Design review of the part shown in the three views and the two pictorial views. Dimensions are in mm from the part's minimum x, y and z. A direction names the side the tool comes from. Coordinates: 2 decimals unless noted, no trailing zeros. Loops run counter-clockwise (first coordinate to the right, second up) from the corner with the lowest first, then second, coordinate; pieces in that order, holes last. Notation, with made-up numbers: (12.25, -6) -> (61.25, -6) arc R19 cw to (61.25, 15) -> close; hole circle Ø10 at (-36.5, 11.5). An arc over 180 degrees is marked (long way). Answer in a Markdown table with one row per item.
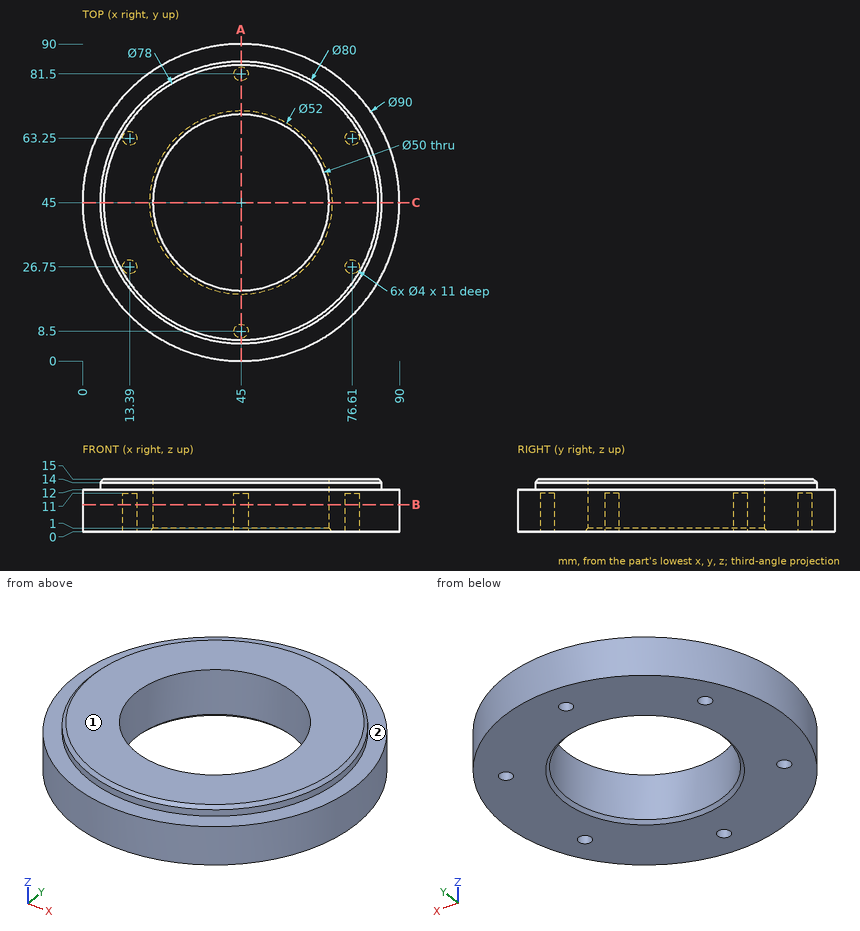
Item 1: Take a section at B-B, the plane z = 7.75. State the section outline as (x, y) points, and give its area (3 significant figures).
Worked answers:
| item | result |
|---|---|
| outline | circle Ø90 at (45, 45); hole circle Ø4 at (13.39, 26.75); hole circle Ø4 at (13.39, 63.25); hole circle Ø50 at (45, 45); hole circle Ø4 at (45, 8.5); hole circle Ø4 at (45, 81.5); hole circle Ø4 at (76.61, 26.75); hole circle Ø4 at (76.61, 63.25) |
| area | 4,320 mm² |
Item 2: Insertion check: pin 1 (3.5 mm diameter, centred on x = 76.61, y = 63.25, fed in from -Z); pin 2 (4 mm diameter, centred on x = 72, z = 2.5, fed in from +Y); pin 3 (8 mm diameter, centred on y = 55.5, z = 8, fed in from -X). Each pin has a flat end and moves straight along its axis. Give the tip position at first contact, or say it passes through.
Worked answers:
| item | result |
|---|---|
| pin 1 | z = 11 |
| pin 2 | y = 82.42 |
| pin 3 | x = 0.47 |
Item 3: Take a section at C-C, the plane y = 45. State the section outline as (x, z) points.
Worked answers:
| item | result |
|---|---|
| outline | (0, 0) -> (19, 0) -> (20, 1) -> (20, 15) -> (6, 15) -> (5, 14) -> (5, 12) -> (0, 12) -> close; (70, 1) -> (71, 0) -> (90, 0) -> (90, 12) -> (85, 12) -> (85, 14) -> (84, 15) -> (70, 15) -> close |
Item 4: For L1, parallel to Y at x = 45, z = 7.75; L2, parallel to X at y = 61.5, z = 8.75; L3, parallel to Z at x = 25, y = 8, list the stretches that pass through material, from the lowest coordinate up.
Worked answers:
| item | result |
|---|---|
| L1 | 0 to 6.5, 10.5 to 20, 70 to 79.5, 83.5 to 90 |
| L2 | 3.13 to 12.42, 14.36 to 26.22, 63.78 to 75.64, 77.58 to 86.87 |
| L3 | 0 to 12 |
Item 5: For the marked faces 1 and 2, list the 3-axis set-ups (+Z, -Z, +X, -X, +Y, -Y) from which the entire face can be reached by the end or side of a thin tool; tool diameter is ignored.
Worked answers:
| item | result |
|---|---|
| face 1 | +Z, +X, -X, +Y, -Y |
| face 2 | +Z |
Item 6: Take a section at A-A, the plane x = 45. State the section outline as (y, z) points.
Worked answers:
| item | result |
|---|---|
| outline | (0, 0) -> (6.5, 0) -> (6.5, 11) -> (10.5, 11) -> (10.5, 0) -> (19, 0) -> (20, 1) -> (20, 15) -> (6, 15) -> (5, 14) -> (5, 12) -> (0, 12) -> close; (70, 1) -> (71, 0) -> (79.5, 0) -> (79.5, 11) -> (83.5, 11) -> (83.5, 0) -> (90, 0) -> (90, 12) -> (85, 12) -> (85, 14) -> (84, 15) -> (70, 15) -> close |
